from build123d import *

# Parameters (mm, degrees)
SKETCH_1_W          = 100
SKETCH_1_H          = 80
EXTRUDE_1_DEPTH     = 2
SKETCH_2_R          = 6.5
CUT_EXTRUDE_1_DEPTH = 2


with BuildPart() as part:
    # 草图1 → 凸台-拉伸1 (new body)
    with BuildSketch(Plane.XY):
        Rectangle(SKETCH_1_W, SKETCH_1_H)
    extrude(amount=EXTRUDE_1_DEPTH)

    # 草图2 → 切除-拉伸1 (cut)
    with BuildSketch(Plane.XY.offset(2)):
        with Locations((-34, 29)):
            Circle(SKETCH_2_R)
        with Locations((34, 29)):
            Circle(SKETCH_2_R)
        with Locations((34, -29)):
            Circle(SKETCH_2_R)
        with Locations((-34, -29)):
            Circle(SKETCH_2_R)
    extrude(amount=-CUT_EXTRUDE_1_DEPTH, mode=Mode.SUBTRACT)


solid = part.part
Check sheet for the modelled part. Datum: model origin and axes. Units: mm. Give positions to 0.01 mm unless a question says otherwise; leave off trailing zeros. Loops run counter-clockwise (first coordinate to the right, second up) from the corner with the lowest first, then second, coordinate; pieces in that order, holes last. Notation, with made-up numbers: M 45,17 L 80,17 A24 ccw 80,51 Z; hole C -4,-22 d3. An arc over 180 degrees is marked long. Return JSON: item names as keys, results as strings. Group by question number.
1. Mould release check, pull along Y, two halves, no side actions. Record for faces 1 (the cylindrical face through (-40.494, -28.714, 1.014)), 2 (the flat face through (-1, 1, 2)), 3 (the flat face through (-1, -40, 1)): released by +Y, released by -Y, zero draft, split by the parting line, or undercut.
2. Thickness scan on L1, parallel to Y at x = -34, z = 1.15; L2, parallel to X at y = -24.5, z = 0.5; L3, parallel to X at y = -26, z = 1.6. Record the ranges inside material, lowest first.
3. Cross-section at C-C on x = -34. Record the boundary of the cut face in (y, z).
4. Go/stop test with flat-tipped pins: pin 1 (11.5 mm diameter, centred on x = -34, y = -29, fed in from -Z); pin 2 (1 mm diameter, centred on x = 9.5, y = -11, fed in from -Z). Record where each tip stops, or that it passes through.
5. Cross-section at A-A on y = -26.5. Record the boundary of the cut face in (x, z), plus the area to 3 significant figures.
6. Cross-section at B-B on z = 0.7. Record the boundary of the cut face in (x, y), plus the area to 3 significant figures.
Return value:
{
 "1": {"face 1": "undercut", "face 2": "zero draft", "face 3": "released by -Y"},
 "2": {"L1": "-40 to -35.5, -22.5 to 22.5, 35.5 to 40", "L2": "-50 to -38.69, -29.31 to 29.31, 38.69 to 50", "L3": "-50 to -39.77, -28.23 to 28.23, 39.77 to 50"},
 "3": {"outline": "M -40,0 L -35.5,0 L -35.5,2 L -40,2 Z; M -22.5,0 L 22.5,0 L 22.5,2 L -22.5,2 Z; M 35.5,0 L 40,0 L 40,2 L 35.5,2 Z"},
 "4": {"pin 1": "through", "pin 2": "z = 0"},
 "5": {"outline": "M -50,0 L -40,0 L -40,2 L -50,2 Z; M -28,0 L 28,0 L 28,2 L -28,2 Z; M 40,0 L 50,0 L 50,2 L 40,2 Z", "area": "152 mm^2"},
 "6": {"outline": "M -50,-40 L 50,-40 L 50,40 L -50,40 Z; hole C -34,-29 d13; hole C -34,29 d13; hole C 34,-29 d13; hole C 34,29 d13", "area": "7,470 mm^2"}
}
